Check sheet for the modelled part. Datum: model origin and axes. Units: mm. Round coordinates to 2 decimals unless told otherwise and drop trailing zeros. Order: outer loops, then holes, each group sorted by start corner. A loop starts at its lowest first (then second) coordinate and runs counter-clockwise, first axis right, second up.
(1) Mould release check, pull along Z, two halves, no side actions. Record for faces 1 (the cylindrical face through (-2, 2, 0)), 2 (the flat face through (0, 0, -21)), 3 (the cylindrical face through (0, 2, -50)), 4 (the cylindrical face through (-0.96, 7.46, -37.69)): released by +Z, released by -Z, zero draft, split by the parting line, or undercut.
(2) Sectioned sample at D-D, the plane y = 7.25. Enter the section's corners in (x, z).
(3) Sectioned sample at B-B, the plane x = 0. Enter the section's corners in (y, z), and give its area (3 significant figures).
(4) Sectioned sample at A-A, the plane z = -41.5. Enter the section's corners in (x, y).
(5) Sectioned sample at C-C, the plane y = 1.5. Enter the section's corners in (x, z).
(6) Thickness scan on probe 1 along Y at (x, z) = (-5.75, -4.5); probe 2 along Z at (x, y) = (1.25, 2.25); probe 3 along Z at (x, y) = (-6.5, 3.5). Record the ranges inside material, lowest first.
(7) Depth check by flat-ended pin: pin 1 (3 mm diameter, centred on x = 3.5, z = -37, fed in from +Y); pin 2 (3 mm diameter, centred on x = -4, y = 2, fed in from -Z); pin 3 (1 mm diameter, centred on x = 5, y = 2.5, fed in from -Z). Enter the tip coordinate at first touch or a pass-through.
```python
from build123d import *

# Parameters (mm, degrees)
SKETCH_1_3_R        = 50
SKETCH_1_3_R_2      = 2.5
BOSS_EXTRUDE1_DEPTH = 5
SKETCH_1_3_2_R      = 2.5
BOSS_EXTRUDE2_DEPTH = 10
CUT_EXTRUDE1_START  = -11
CUT_EXTRUDE1_DEPTH  = 11
SKETCH2_R           = 2
CUT_EXTRUDE2_DEPTH  = 52.789634215


with BuildPart() as part:
    # Sketch 1_3 → Boss-Extrude1 (new body)
    # profile 1 of 2: a face of its own
    with BuildSketch(Plane(origin=(0, 0, 0), x_dir=(1, 0, 0), z_dir=(0, 1, 0))):
        with Locations(Location((0, 0, 0), (0, 0, 270))):
            Circle(SKETCH_1_3_R)
        with Locations((0, 40)):
            Circle(SKETCH_1_3_R_2, mode=Mode.SUBTRACT)
    # profile 2 of 2: a face of its own
    with BuildSketch(Plane(origin=(0, 0, 0), x_dir=(1, 0, 0), z_dir=(0, 1, 0))):
        with Locations((0, 40)):
            Circle(SKETCH_1_3_R_2)
    extrude(amount=BOSS_EXTRUDE1_DEPTH)

    # Sketch 1_3 2 → Boss-Extrude2 (add)
    with BuildSketch(Plane(origin=(0, 0, 0), x_dir=(1, 0, 0), z_dir=(0, 1, 0))):
        with Locations(Location((0, 40, 0), (0, 0, 270))):
            Circle(SKETCH_1_3_2_R)
    extrude(amount=BOSS_EXTRUDE2_DEPTH)

    # Sketch5 → Cut-Extrude1 (cut)
    with BuildSketch(Plane(origin=(0, 5, 0), x_dir=(1, 0, 0), z_dir=(0, 1, 0)).offset(CUT_EXTRUDE1_START)):
        with BuildLine():
            Line((9.064558023, 20), (9.064558023, 0))
            ThreePointArc((9.064558023, 0), (0, -9.064558023), (-9.064558023, 0))
            Line((-9.064558023, 0), (-9.064558023, 20))
            Line((-9.064558023, 20), (-9.064558023, 49.171473314))
            ThreePointArc((-9.064558023, 49.171473314), (0, -50), (9.064558023, 49.171473314))
            Line((9.064558023, 49.171473314), (9.064558023, 20))
        make_face()
    extrude(amount=CUT_EXTRUDE1_DEPTH, mode=Mode.SUBTRACT)

    # Sketch2 → Cut-Extrude2 (cut, through all)
    with BuildSketch(Plane.XZ):
        with Locations(Location((0, 0, 0), (0, 0, 270))):
            Circle(SKETCH2_R)
    extrude(amount=-CUT_EXTRUDE2_DEPTH, mode=Mode.SUBTRACT)


solid = part.part
```
Derived:
1. face 1: undercut
1. face 2: zero draft
1. face 3: released by -Z
1. face 4: split by the parting line
2. outline: circle Ø5 at (0, -40)
3. outline: (0, -50) - (5, -50) - (5, -42.5) - (10, -42.5) - (10, -37.5) - (5, -37.5) - (5, -2) - (0, -2) - close; (0, 2) - (5, 2) - (5, 9.06) - (0, 9.06) - close
3. area: 300 mm2
4. outline: (-9.06, 0) - (9.06, 0) - (9.06, 5) - (2, 5) - (2, 10) - (-2, 10) - (-2, 5) - (-9.06, 5) - close
5. outline: (-9.06, -49.17) arc R50 ccw to (9.06, -49.17) - (9.06, 0) arc R9.06 ccw to (-9.06, 0) - close; hole circle Ø4 at (0, 0)
6. probe 1: y = 0 to 5
6. probe 2: z = -49.98 to -1.56, 1.56 to 8.98
6. probe 3: z = -49.58 to 6.32
7. pin 1: stops at y = 5
7. pin 2: stops at z = -49.94
7. pin 3: stops at z = -49.8
